Work out the finished part from the listing and answer in its coordinate system (mm). Coordinates: 2 decimals unless noted, no trailing zeros. Order: outer loops, then holes, each group sorted by start corner. A loop starts at its lowest first (then second) coordinate and runs counter-clockwise, first axis right, second up.
1. The part is cut by section C-C, the plane z = -462.5. Give the vertices of the cut face in (x, y).
2. A flat-ended cylindrical pin translates along its axis: pin 1 Ø6 at (x, y) = (8.5, -21) entering from -Z. Find the tip coordinate at first contact, or state that the pin passes through.
3. Find the intervals of material crossed by probe 1 along X at (y, z) = (12, 955.5); probe 2 along X at (y, z) = (-24.5, -632.5), in increasing order.
4. The part is cut by section A-A, the plane x = 6. Give the vertices of the cut face in (y, z).
```python
from build123d import *

# Parameters (mm, degrees)
SKETCH1_W           = 60
SKETCH1_H           = 60
SKETCH1_W_2         = 52
SKETCH1_H_2         = 52
BOSS_EXTRUDE1_DEPTH = 1165
FILLET1_R           = 6
FILLET2_R           = 3


with BuildPart() as part:
    # Sketch1 → Boss-Extrude1 (new, symmetric)
    with BuildSketch(Plane.XY):
        Rectangle(SKETCH1_W, SKETCH1_H)
        Rectangle(SKETCH1_W_2, SKETCH1_H_2, mode=Mode.SUBTRACT)
    extrude(amount=BOSS_EXTRUDE1_DEPTH, both=True)

    # Fillet1
    fillet1_edges = [part.edges().sort_by_distance(p)[0] for p in [
        (30, -30, 0),
        (-30, -30, 0),
        (-30, 30, 0),
        (30, 30, 0),
    ]]
    fillet(fillet1_edges, radius=FILLET1_R)

    # Fillet2
    fillet2_edges = [part.edges().sort_by_distance(p)[0] for p in [
        (26, -26, 0),
        (26, 26, 0),
        (-26, 26, 0),
        (-26, -26, 0),
    ]]
    fillet(fillet2_edges, radius=FILLET2_R)


solid = part.part
```
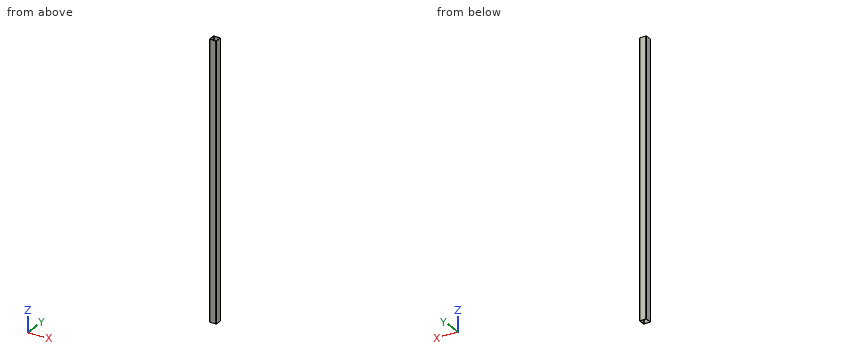
Geometry says:
1. outline: (-30, -24) arc R6 ccw to (-24, -30) - (24, -30) arc R6 ccw to (30, -24) - (30, 24) arc R6 ccw to (24, 30) - (-24, 30) arc R6 ccw to (-30, 24) - close; hole (-26, -23) arc R3 ccw to (-23, -26) - (23, -26) arc R3 ccw to (26, -23) - (26, 23) arc R3 ccw to (23, 26) - (-23, 26) arc R3 ccw to (-26, 23) - close
2. pin 1: passes through
3. probe 1: x = -30 to -26, 26 to 30
3. probe 2: x = -29.98 to -25.6, 25.6 to 29.98
4. outline: (-30, -1165) - (-26, -1165) - (-26, 1165) - (-30, 1165) - close; (26, -1165) - (30, -1165) - (30, 1165) - (26, 1165) - close
